Read the model definition and answer for the solid it produces. Units are mm, in the model's axes. A direction names the side the tool comes from. Give positions to 0.01 mm unless a question says otherwise; leave off trailing zeros. Write each loop counter-clockwise with the first axis right and the second up, starting at its lowest first coordinate (ties: lowest second). Pieces come first, ordered by that corner, then holes.
```python
from build123d import *

# Parameters (mm, degrees)
SKETCH1_R                   = 74
BOSS_EXTRUDE1_DEPTH         = 65
FILLET1_R                   = 10
SKETCH2_R                   = 10
BOSS_EXTRUDE2_DEPTH         = 15
BOSS_EXTRUDE3_START         = -200
SKETCH3_W                   = 194.285714286
SKETCH3_H                   = 160
SKETCH3_R                   = 4
BOSS_EXTRUDE3_DEPTH         = 15
BOSS_EXTRUDE4_DEPTH         = 10
SKETCH5_R                   = 10
BOSS_EXTRUDE5_DEPTH         = 90
SKETCH6_R                   = 3
BOSS_EXTRUDE6_DEPTH         = 80
SKETCH7_R                   = 7.5
BOSS_EXTRUDE7_DEPTH         = 12
SKETCH8_R                   = 5.5
BOSS_EXTRUDE8_DEPTH         = 3
CHAMFER1_SIZE               = 2
M5_TAPPED_HOLE1_D           = 4.2
M5_TAPPED_HOLE1_DEPTH       = 14
M5_TAPPED_HOLE1_CSINK_D     = 5.05
M5_TAPPED_HOLE1_CSINK_ANGLE = 90
M5_TAPPED_HOLE1_TIP         = 1.2618073


with BuildPart() as part:
    # Sketch1 → Boss-Extrude1 (new, symmetric)
    with BuildSketch(Plane.XY):
        Circle(SKETCH1_R)
    extrude(amount=BOSS_EXTRUDE1_DEPTH, both=True)

    # Fillet1
    fillet1_edges = [part.edges().sort_by_distance(p)[0] for p in [
        (-74, 0, -65),
        (-74, 0, 65),
    ]]
    fillet(fillet1_edges, radius=FILLET1_R)

    # Sketch2 → Boss-Extrude2 (add)
    with BuildSketch(Plane.XY.offset(65)):
        Circle(SKETCH2_R)
    extrude(amount=BOSS_EXTRUDE2_DEPTH)



with BuildPart() as body_2:
    # Sketch3 → Boss-Extrude3 (new body)
    with BuildSketch(Plane.XY.offset(80).offset(BOSS_EXTRUDE3_START)):
        Rectangle(SKETCH3_W, SKETCH3_H)
        with Locations((-85, 70)):
            Circle(SKETCH3_R, mode=Mode.SUBTRACT)
        with Locations((85, 70)):
            Circle(SKETCH3_R, mode=Mode.SUBTRACT)
        with Locations((85, -70)):
            Circle(SKETCH3_R, mode=Mode.SUBTRACT)
        with Locations((-85, -70)):
            Circle(SKETCH3_R, mode=Mode.SUBTRACT)
    extrude(amount=BOSS_EXTRUDE3_DEPTH)

    # Sketch4 → Boss-Extrude4 (add)
    with BuildSketch(Plane.ZY.offset(97.142857143)):
        Polygon((-105, 62.5), (20, 35), (20, -35), (-105, -62.5), align=None)
    boss_extrude4 = extrude(amount=-BOSS_EXTRUDE4_DEPTH)

    # Mirror1: Boss-Extrude4 across plane
    add(boss_extrude4.mirror(Plane(origin=(0, 0, 0), x_dir=(0, 0, 1), z_dir=(1, 0, 0))))


with BuildPart() as part_1:
    add(part.part)

    add(body_2.part)  # Boss-Extrude5 merges body 2
    # Sketch5 → Boss-Extrude5 (add, symmetric)
    with BuildSketch(Plane(origin=(0, 0, 0), x_dir=(0, 0, -1), z_dir=(1, 0, 0))):
        with Locations(Location((0, 0, 0), (0, 0, 180))):
            Circle(SKETCH5_R)
    extrude(amount=BOSS_EXTRUDE5_DEPTH, both=True)

    # Sketch6 → Boss-Extrude6 (add)
    with BuildSketch(Plane.XY.offset(80)):
        Circle(SKETCH6_R)
    extrude(amount=BOSS_EXTRUDE6_DEPTH)

    # Sketch7 → Boss-Extrude7 (add)
    with BuildSketch(Plane.XY.offset(160)):
        Circle(SKETCH7_R)
    extrude(amount=BOSS_EXTRUDE7_DEPTH)

    # Sketch8 → Boss-Extrude8 (add)
    with BuildSketch(Plane.XY.offset(172)):
        Circle(SKETCH8_R)
    extrude(amount=BOSS_EXTRUDE8_DEPTH)

    # Chamfer1
    chamfer1_edges = [part_1.edges().sort_by_distance(p)[0] for p in [
        (-5.5, 0, 175),
    ]]
    chamfer(chamfer1_edges, length=CHAMFER1_SIZE)

    # M5 Tapped Hole1
    with Locations(Plane.XY.offset(175)):
        with Locations((0, 0)):
            CounterSinkHole(M5_TAPPED_HOLE1_D / 2, M5_TAPPED_HOLE1_CSINK_D / 2, depth=M5_TAPPED_HOLE1_DEPTH, counter_sink_angle=M5_TAPPED_HOLE1_CSINK_ANGLE)
            with Locations((0, 0, -(M5_TAPPED_HOLE1_DEPTH + M5_TAPPED_HOLE1_TIP / 2))):  # 118° drill point
                Cone(0, M5_TAPPED_HOLE1_D / 2, M5_TAPPED_HOLE1_TIP, mode=Mode.SUBTRACT)


solid = part_1.part
```
Item 1: Section A-A (z = -100.5) is taken. Write down the section's boundary in (x, y), and give its area (3 significant figures).
Result set:
outline: (-97.14, -61.51) - (-87.14, -61.51) - (-87.14, 61.51) - (-97.14, 61.51) - close; (87.14, -61.51) - (97.14, -61.51) - (97.14, 61.51) - (87.14, 61.51) - close
area: 2,460 mm2
Item 2: Which of the six approach directions +Z, -Z, +X, -X, +Y, -Y give full straight-line access (tool end or side, diameter ignored) to faces 4 (the flat face through (92.21, 48.94, -43.37)), 5 (the flat face through (-92, 0, 20)), 6 (the flat face through (92, 0, 20)), 7 (the cylindrical face through (-7.493, 0.33, 165.916)), 8 (the flat face through (-92.21, -48.56, -41.63))?
Result set:
face 4: +Z, +X, +Y
face 5: +Z, -X, +Y, -Y
face 6: +Z, +X, +Y, -Y
face 7: +Z
face 8: +Z, -X, -Y
Item 3: Find the intervals of material crossed by line 1 along Y through (x, z) = (-85, -111.5); line 2 along X through (y, z) = (2, -49); line 3 along Z through (x, y) = (-15, 57), in increasing order.
Result set:
line 1: y = -80 to -74, -66 to 66, 74 to 80
line 2: x = -97.14 to -87.14, -73.97 to 73.97, 87.14 to 97.14
line 3: z = -120 to -105, -65 to 65
Item 4: Section B-B (z = -21.5) is taken. Write down the section's boundary in (x, y).
Result set:
outline: (-97.14, -44.13) - (-87.14, -44.13) - (-87.14, 44.13) - (-97.14, 44.13) - close; circle Ø148 at (0, 0); (87.14, -44.13) - (97.14, -44.13) - (97.14, 44.13) - (87.14, 44.13) - close
Item 5: Determine the mould class of faces 1 (the flat face through (3.2, 0.1, 160)), 2 (the cylindrical face through (-85.867, 66.095, -112.605)), 3 (the flat face through (-92.21, 48.94, -43.37)) for opening direction Z: pulls with the +Z half, pulls with the -Z half, needs draft (parallel to the pull), parting line crosses it, or undercut.
Result set:
face 1: undercut
face 2: needs draft
face 3: pulls with the +Z half
Item 6: Each of these flat-tipped pins is pushed along its axis until it touches: pin 1 Ø10 at (y, z) = (-61, 0.5) entering from +X; pin 2 Ø10.5 at (x, y) = (-85, -70) entering from +Z; pin 3 Ø1.5 at (x, z) = (75, -50) entering from +Y; pin 4 Ø1.5 at (x, z) = (-3.5, -13) entering from -Y. Where does it stop, or does it pass through?
Result set:
pin 1: stops at x = 48.37
pin 2: stops at z = -105
pin 3: passes through
pin 4: stops at y = -73.95
